Geometry: final body of the model. Coordinates: model frame, mm. A direction names the side the tool comes from. Round coordinates to 2 decimals unless told otherwise and drop trailing zeros. Loops run counter-clockwise (first coordinate to the right, second up) from the corner with the lowest first, then second, coordinate; pieces in that order, holes last. Notation, with made-up numbers: (16, 43.25) - (58, 43.25) arc R32 ccw to (58, 70.25) - close; hole circle Ø4 at (75.25, 66). An arc over 180 degrees is marked (long way). Return JSON: item names as keys, results as strings. Group by question number.
1. Material intervals for probe 1 along X at (y, z) = (14, 502.5); probe 2 along Y at (x, z) = (7.5, 1556.5), sorted ascending.
2. First-contact query: pin 1 Ø9 at (y, z) = (23.5, 580) entering from +X; pin 2 Ø3 at (x, z) = (21, 303.5) entering from +Y; pin 3 Ø2 at (x, z) = (9, 227) entering from +Y. Flat tips, straight axial feed; report the tip coordinate or a pass-through.
3. Section B-B on x = 22.5. Return loops of the section in (y, z).
4. Set-up query: faces 1 (the face through (24, 4, 838)), 2 (the face through (20, 0, 838)). Return all of +Z, -Z, +X, -X, +Y, -Y with unobstructed straight access to the full face (end or side cutting, diameter ignored); none if empty.
5. Section A-A on z = 267. Return loops of the section in (x, y).
from build123d import *

# Parameters (mm, degrees)
BOSS_EXTRUDE1_DEPTH = 1700


with BuildPart() as part:
    # Sketch1 → Boss-Extrude1 (new body)
    with BuildSketch(Plane.XY):
        with BuildLine():
            Line((0, 0), (0, 40))
            Line((0, 40), (2.666666667, 40))
            ThreePointArc((2.666666667, 40), (3.609475708, 39.609475708), (4, 38.666666667))
            Line((4, 38.666666667), (4, 9))
            ThreePointArc((4, 9), (5.464466094, 5.464466094), (9, 4))
            Line((9, 4), (38.666666667, 4))
            ThreePointArc((38.666666667, 4), (39.609475708, 3.609475708), (40, 2.666666667))
            Line((40, 2.666666667), (40, 0))
            Line((40, 0), (0, 0))
        make_face()
    extrude(amount=BOSS_EXTRUDE1_DEPTH)


solid = part.part
Taken from the geometry:
{
 "1": {"probe 1": "0 to 4", "probe 2": "0 to 4.23"},
 "2": {"pin 1": "x = 4", "pin 2": "y = 4", "pin 3": "y = 4.1"},
 "3": {"outline": "(0, 0) - (4, 0) - (4, 1700) - (0, 1700) - close"},
 "4": {"face 1": "+Z, -Z, +X, +Y", "face 2": "+Z, -Z, +X, -X, -Y"},
 "5": {"outline": "(0, 0) - (40, 0) - (40, 2.67) arc R1.33 ccw to (38.67, 4) - (9, 4) arc R5 cw to (4, 9) - (4, 38.67) arc R1.33 ccw to (2.67, 40) - (0, 40) - close"}
}
